```python
from build123d import *

# Parameters (mm, degrees)
SKETCH_1_W              = 130
SKETCH_1_H              = 130
EXTRUDE_1_DEPTH         = 4
CHAMFER_1_SIZE          = 2
HOLE_WIZARD_13_0_13_1_D = 13


with BuildPart() as part:
    # 草图1 → 凸台-拉伸1 (new body)
    with BuildSketch(Plane.XY):
        with Locations((-65, 0)):
            Rectangle(SKETCH_1_W, SKETCH_1_H)
    extrude(amount=EXTRUDE_1_DEPTH)

    # 倒角1
    chamfer_1_edges = [part.edges().sort_by_distance(p)[0] for p in [
        (0, -65, 2),
        (-130, -65, 2),
        (-130, 65, 2),
        (0, 65, 2),
    ]]
    chamfer(chamfer_1_edges, length=CHAMFER_1_SIZE)

    # Ø13.0 (13) 直径孔1 (through all)
    with Locations(Plane(origin=(0, 0, 0), x_dir=(-1, 0, 0), z_dir=(0, 0, -1))):
        with Locations((15, -50), (15, 50), (115, -50), (115, 50)):
            Hole(HOLE_WIZARD_13_0_13_1_D / 2)


solid = part.part
```
Check sheet for the modelled part. Datum: model origin and axes. Units: mm. Round coordinates to 2 decimals unless told otherwise and drop trailing zeros. Write each loop counter-clockwise with the first axis right and the second up, starting at its lowest first coordinate (ties: lowest second). Pieces come first, ordered by that corner, then holes. Notation, with made-up numbers: (-37.5, 81) -> (17.5, 81) arc R19 ccw to (17.5, 115) -> close; hole circle Ø7 at (-35.75, 59.25). An arc over 180 degrees is marked (long way). Put each result on its own line as item: value.
(1) Sectioned sample at C-C (z = 2.75). Enter the section's corners in (x, y).
Values found:
outline: (-130, -63) -> (-128, -65) -> (-2, -65) -> (0, -63) -> (0, 63) -> (-2, 65) -> (-128, 65) -> (-130, 63) -> close; hole circle Ø13 at (-115, -50); hole circle Ø13 at (-115, 50); hole circle Ø13 at (-15, -50); hole circle Ø13 at (-15, 50)
(2) Sectioned sample at A-A (y = -50). Enter the section's corners in (x, z), plus the area to 3 significant figures.
Values found:
outline: (-130, 0) -> (-121.5, 0) -> (-121.5, 4) -> (-130, 4) -> close; (-108.5, 0) -> (-21.5, 0) -> (-21.5, 4) -> (-108.5, 4) -> close; (-8.5, 0) -> (0, 0) -> (0, 4) -> (-8.5, 4) -> close
area: 416 mm^2
(3) Sectioned sample at B-B (x = -115). Enter the section's corners in (y, z), plus the area to 3 significant figures.
Values found:
outline: (-65, 0) -> (-56.5, 0) -> (-56.5, 4) -> (-65, 4) -> close; (-43.5, 0) -> (43.5, 0) -> (43.5, 4) -> (-43.5, 4) -> close; (56.5, 0) -> (65, 0) -> (65, 4) -> (56.5, 4) -> close
area: 416 mm^2
(4) Mould release check, pull along X, two halves, no side actions. Record for faces 1 (the face through (-130, -1, 2)), 2 (the face through (-66, 1, 4)), 3 (the face through (-121.494, 50.286, 2.028)), 4 (the face through (-20.158, -53.955, 2.028)): released by +X, released by -X, zero draft, split by the parting line, or undercut.
Values found:
face 1: released by -X
face 2: zero draft
face 3: undercut
face 4: undercut
(5) Material ranges on line 1 (Y direction, x = -115, z = 2.05); line 2 (Y direction, x = -119.5, z = 3.75); line 3 (X direction, y = -55.5, z = 3.6), recorded low to high.
Values found:
line 1: y = -65 to -56.5, -43.5 to 43.5, 56.5 to 65
line 2: y = -65 to -54.69, -45.31 to 45.31, 54.69 to 65
line 3: x = -130 to -118.46, -111.54 to -18.46, -11.54 to 0
